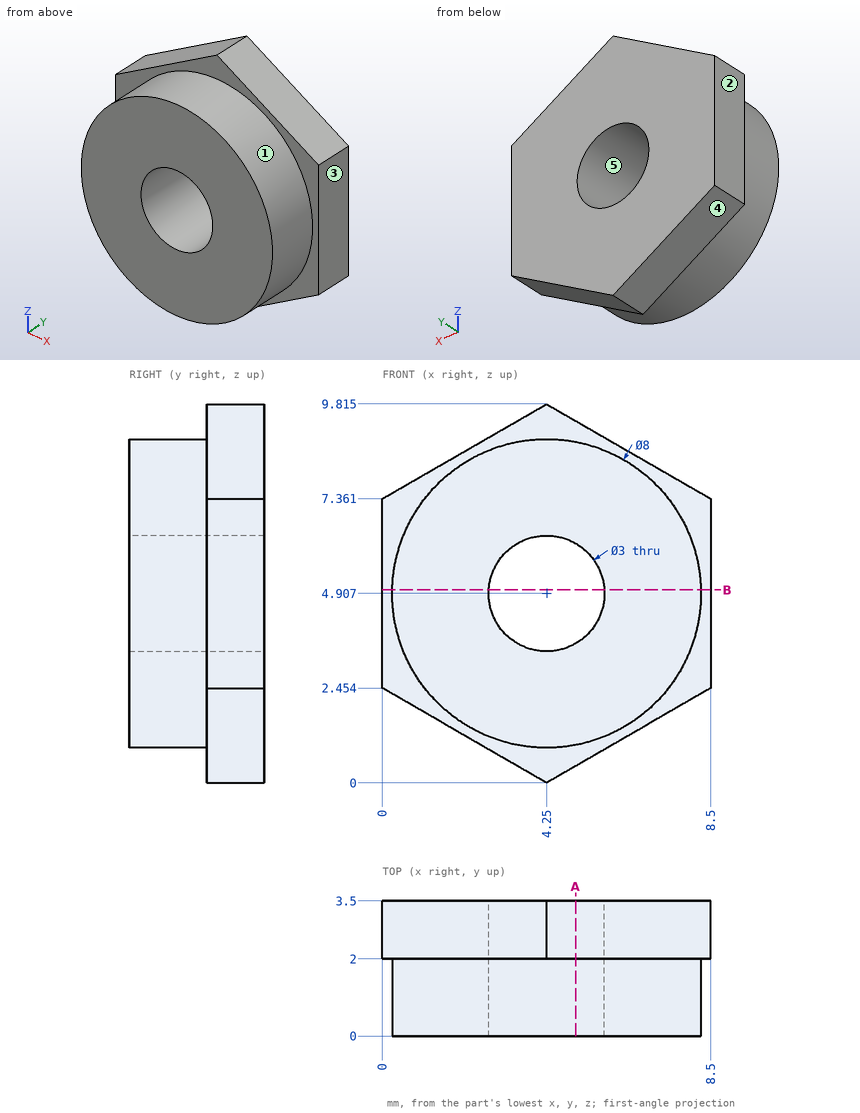
Verification items for this drawing (mm, ordinates from the low corner). A direction names the side the tool comes from. Round coordinates to 2 decimals unless told otherwise and drop trailing zeros. Loops run counter-clockwise (first coordinate to the right, second up) from the corner with the lowest first, then second, coordinate; pieces in that order, holes last. Notation, with made-up numbers: (7.25, 7.25) - (50.25, 7.25) arc R28 cw to (50.25, 30.25) - close; hole circle Ø10 at (-19, -33.75). An arc over 180 degrees is marked (long way). Write item = value, one per line.
Q1. Sectioned sample at A-A on x = 5. Record the boundary of the cut face in (y, z).
Here are the results:
outline = (0, 0.98) - (2, 0.98) - (2, 0.43) - (3.5, 0.43) - (3.5, 3.61) - (0, 3.61) - close; (0, 6.21) - (3.5, 6.21) - (3.5, 9.38) - (2, 9.38) - (2, 8.84) - (0, 8.84) - close
Q2. Tool access check on the marked faces 1 and 2. Record the directions out of +Z, -Z, +X, -X, +Y, -Y that give a thin tool (end or side, any length) a straight path to the whole face; none if there is none.
Here are the results:
face_1 = -Y
face_2 = +Z, -Z, -X, +Y, -Y
Q3. Depth check by flat-ended pin: pin 1 (2 mm diameter, centred on x = 2, y = 0.5, fed in from +Z); pin 2 (2 mm diameter, centred on x = 6, z = 2.5, fed in from -Y); pin 3 (1.8 mm diameter, centred on x = 4.25, z = 4.91, fed in from +Y) (1 decimal); pin 4 (2 mm diameter, centred on y = 2.5, z = 8.5, fed in from -X). Enter the tip coordinate at first touch or a pass-through.
Here are the results:
pin_1 = 8.71
pin_2 = 0
pin_3 = through
pin_4 = 0.24
Q4. Sectioned sample at B-B on z = 5. Record the boundary of the cut face in (x, y).
Here are the results:
outline = (0, 2) - (0.25, 2) - (0.25, 0) - (2.75, 0) - (2.75, 3.5) - (0, 3.5) - close; (5.75, 0) - (8.25, 0) - (8.25, 2) - (8.5, 2) - (8.5, 3.5) - (5.75, 3.5) - close
Q5. Mould release check, pull along X, two halves, no side actions. Record for the marked faces 3, 4 and 5: +X half, -X half, draft (parallel to the pull), parting line (faces both ways), or undercut.
Here are the results:
face_3 = +X half
face_4 = -X half
face_5 = undercut
Q6. Material ranges on L1, parallel to Y at x = 6.25, z = 8.5; L2, parallel to Z at x = 6.75, y = 0.6 (1 decimal); L3, parallel to X at y = 2.2, z = 4.75, recorded low to high.
Here are the results:
L1 = 2 to 3.5
L2 = 1.8 to 8
L3 = 0 to 2.76, 5.74 to 8.5
